Source: CAD feature listing. Evaluate the final solid. Frame: model axes, mm. Round coordinates to 2 decimals unless told otherwise and drop trailing zeros. Order: outer loops, then holes, each group sorted by start corner. A loop starts at its lowest first (then second) coordinate and runs counter-clockwise, first axis right, second up.
```python
from build123d import *

# Parameters (mm, degrees)
BOSS_EXTRUDE1_DEPTH = 337.5


with BuildPart() as part:
    # Sketch1 → Boss-Extrude1 (new, symmetric)
    with BuildSketch(Plane.XY):
        with BuildLine():
            Line((0, 0), (0, 30))
            Line((0, 30), (2, 30))
            ThreePointArc((2, 30), (2.707106781, 29.707106781), (3, 29))
            Line((3, 29), (3, 7.5))
            ThreePointArc((3, 7.5), (4.318019485, 4.318019485), (7.5, 3))
            Line((7.5, 3), (29, 3))
            ThreePointArc((29, 3), (29.707106781, 2.707106781), (30, 2))
            Line((30, 2), (30, 0))
            Line((30, 0), (0, 0))
        make_face()
    extrude(amount=BOSS_EXTRUDE1_DEPTH, both=True)


solid = part.part
```
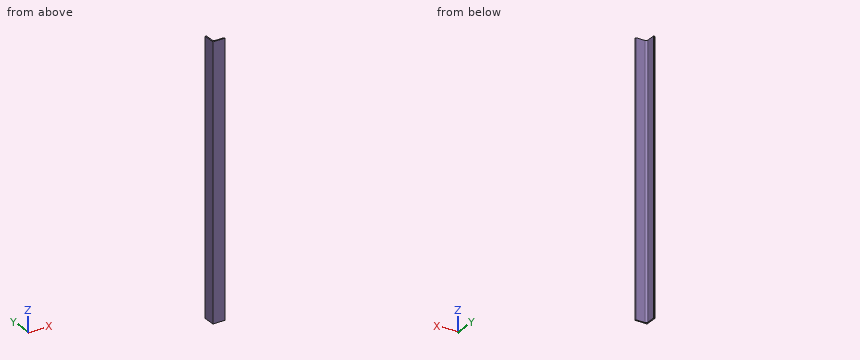
1. First-contact query: pin 1 (17 mm diameter, centred on x = 14, z = 68.5, fed in from +Y); pin 2 (1 mm diameter, centred on y = 6.5, z = 113.5, fed in from +X); pin 3 (11 mm diameter, centred on y = 18.5, z = -91.5, fed in from +X). Flat tips, straight axial feed; report the tip coordinate or a pass-through.
2. Line query: line 1 along Y through (x, z) = (12, 136); line 2 along Y through (x, z) = (6, -175.5). Output: solid intervals per line, ascending.
3. Section A-A on z = -3.5. Return loops of the section in (x, y).
4. Section B-B on y = 16.5. Return loops of the section in (x, z), plus the area to 4 significant figures.
Result:
1. pin 1: stops at y = 3.47
1. pin 2: stops at x = 3.26
1. pin 3: stops at x = 3
2. line 1: y = 0 to 3
2. line 2: y = 0 to 3.26
3. outline: (0, 0) - (30, 0) - (30, 2) arc R1 ccw to (29, 3) - (7.5, 3) arc R4.5 cw to (3, 7.5) - (3, 29) arc R1 ccw to (2, 30) - (0, 30) - close
4. outline: (0, -337.5) - (3, -337.5) - (3, 337.5) - (0, 337.5) - close
4. area: 2,025 mm2
